Design review of the part built by this model. Coordinates are the model's own, in mm. A direction names the side the tool comes from. Coordinates: 2 decimals unless noted, no trailing zeros. Loops run counter-clockwise (first coordinate to the right, second up) from the corner with the lowest first, then second, coordinate; pieces in that order, holes last. Notation, with made-up numbers: (-9.5, -1) - (-1.5, -1) arc R22 ccw to (-1.5, 10) - close; hole circle Ø2 at (25, -11.5). An arc over 180 degrees is marked (long way). Use one line per item in the form item = value. Start each with the question number.
(1) Clearance check with flat-ended pins moving along their axes: pin 1 Ø2 at (x, y) = (21.5, -27.5) entering from +Z; pin 2 Ø6 at (x, z) = (13.5, 698) entering from -Y; pin 3 Ø1 at (y, z) = (-2.5, 1059.5) entering from -X. State where each tip first meets the part, or that it passes through.
(2) The part is to be moulded in two halves that separate along Z. For faces 1 (the face through (18, -36, 875)), 2 (the face through (-5, 16, 1467)), 3 (the face through (-47.954, 2.11, 404.58)), say which applies: pulls with the +Z half, pulls with the -Z half, needs draft (parallel to the pull), parting line crosses it, or undercut.
(3) Add section A-A (z = 1293.5). State the section outline as (x, y) points, plus the area to 3 significant figures.
(4) For L1, parallel to Z at x = -39, y = 2; L2, parallel to Z at x = 22, y = -11.5; L3, parallel to X at y = 1.5, z = 1369, list the stretches that pass through material, from the lowest coordinate up.
(5) Tool access review of faces 4 (the face through (-47.954, 2.11, 1004.58)), 5 (the face through (1, 13, 1477)), 6 (the face through (18, -36, 935)): name each direction out of +Z, -Z, +X, -X, +Y, -Y from which nothing blocks a thin tool from reaching the whole face with its end or side.
```python
from build123d import *

# Parameters (mm, degrees)
SKETCH_1_R             = 48
EXTRUDE_1_DEPTH        = 1410
SKETCH_2_R             = 16
EXTRUDE_2_DEPTH        = 67
EXTRUDE_START          = 67
SKETCH_3_R             = 16
EXTRUDE_3_DEPTH        = 67
SKETCH_4_R             = 12.5
EXTRUDE_4_DEPTH        = 80
EXTRUDE_START_2        = 35
SKETCH_5_R             = 12.5
EXTRUDE_5_DEPTH        = 35
SKETCH_6_OUTSIDE_W     = 430.91
SKETCH_6_OUTSIDE_H     = 430.91
SKETCH_6_OUTSIDE_R     = 10
CUT_EXTRUDE_1_DEPTH    = 30
SKETCH_7_W             = 40
SKETCH_7_H             = 8
PATTERN_LINEAR_1_COUNT = 14
PATTERN_LINEAR_1_PITCH = 100
SKETCH_9_R             = 25
EXTRUDE_6_DEPTH        = 57
EXTRUDE_START_3        = 57
SKETCH_10_R            = 25
EXTRUDE_7_DEPTH        = 57
CHAMFER_1_SIZE         = 0.5


with BuildPart() as part:
    # 草图1 → 凸台-拉伸1 (new body)
    with BuildSketch(Plane.XY):
        Circle(SKETCH_1_R)
    extrude(amount=EXTRUDE_1_DEPTH)

    # 草图2 → 凸台-拉伸2 (add)
    with BuildSketch(Plane.XY.offset(1410)):
        Circle(SKETCH_2_R)
    extrude(amount=EXTRUDE_2_DEPTH)

    # 草图3 → 凸台-拉伸3 (add)
    with BuildSketch(Plane(origin=(0, 0, 0), x_dir=(-1, 0, 0), z_dir=(0, 0, -1)).offset(EXTRUDE_START)):
        with Locations(Location((0, 0, 0), (0, 0, 180))):
            Circle(SKETCH_3_R)
    extrude(amount=-EXTRUDE_3_DEPTH)

    # 草图4 → 凸台-拉伸4 (add)
    with BuildSketch(Plane(origin=(0, 0, -67), x_dir=(-1, 0, 0), z_dir=(0, 0, -1))):
        Circle(SKETCH_4_R)
    extrude(amount=EXTRUDE_4_DEPTH)

    # 草图5 → 凸台-拉伸5 (add)
    with BuildSketch(Plane.XY.offset(1477).offset(EXTRUDE_START_2)):
        with Locations(Location((0, 0, 0), (0, 0, 180))):
            Circle(SKETCH_5_R)
    extrude(amount=-EXTRUDE_5_DEPTH)

    # 草图6 outside → 切除-拉伸1 (cut)
    with BuildSketch(Plane(origin=(0, 0, -147), x_dir=(-1, 0, 0), z_dir=(0, 0, -1))):
        Rectangle(SKETCH_6_OUTSIDE_W, SKETCH_6_OUTSIDE_H)
        Circle(SKETCH_6_OUTSIDE_R, mode=Mode.SUBTRACT)
    extrude(amount=-CUT_EXTRUDE_1_DEPTH, mode=Mode.SUBTRACT)

    # 草图7 → 切除-旋转1 (revolve, cut)
    with BuildSketch(Plane(origin=(0, 0, 0), x_dir=(0, 0, -1), z_dir=(1, 0, 0)), mode=Mode.PRIVATE) as cut_revolve_1_sk:
        with Locations((-55, -44)):
            Rectangle(SKETCH_7_W, SKETCH_7_H)
    cut_revolve_1 = revolve(cut_revolve_1_sk.sketch.rotate(Axis((0, 0, 0), (0, 0, 1)), 270), axis=Axis((0, 0, 0), (0, 0, 1)), mode=Mode.SUBTRACT)

    # 阵列(线性)1: 切除-旋转1 ×14
    with Locations(*[(0, 0, i * PATTERN_LINEAR_1_PITCH) for i in range(1, PATTERN_LINEAR_1_COUNT)]):
        add(cut_revolve_1, mode=Mode.SUBTRACT)

    # 草图9 → 凸台-拉伸6 (add)
    with BuildSketch(Plane.XY.offset(1410)):
        with Locations(Location((0, 0, 0), (0, 0, 180))):
            Circle(SKETCH_9_R)
    extrude(amount=EXTRUDE_6_DEPTH)

    # 草图10 → 凸台-拉伸7 (add)
    with BuildSketch(Plane(origin=(0, 0, 0), x_dir=(-1, 0, 0), z_dir=(0, 0, -1)).offset(EXTRUDE_START_3)):
        Circle(SKETCH_10_R)
    extrude(amount=-EXTRUDE_7_DEPTH)

    # 倒角1
    chamfer_1_edges = [part.edges().sort_by_distance(p)[0] for p in [
        (-16, 0, -67),
        (25, 0, 1467),
        (25, 0, -57),
        (12.5, 0, 1512),
        (12.5, 0, -117),
        (10, 0, -147),
        (-16, 0, 1477),
    ]]
    chamfer(chamfer_1_edges, length=CHAMFER_1_SIZE)


solid = part.part
```
Computed values:
q1.pin_1 = 1410
q1.pin_2 = -46.84
q1.pin_3 = -39.95
q2.face_1 = undercut
q2.face_2 = pulls with the +Z half
q2.face_3 = needs draft
q3.outline = circle Ø96 at (0, 0)
q3.area = 7,240 mm^2
q4.L1 = 0 to 1410
q4.L2 = -56.68 to 1466.68
q4.L3 = -39.97 to 39.97
q5.face_4 = +Z, -Z
q5.face_5 = +Z
q5.face_6 = none
